```python
from build123d import *

# Parameters (mm, degrees)
SKETCH1_R           = 13
SKETCH1_R_2         = 6.25
BOSS_EXTRUDE1_DEPTH = 9


with BuildPart() as part:
    # Sketch1 → Boss-Extrude1 (new body)
    with BuildSketch(Plane(origin=(0, 0, 0), x_dir=(1, 0, 0), z_dir=(0, 1, 0))):
        with BuildLine():
            Line((2.928932188, 22.071067812), (22.071067812, 2.928932188))
            ThreePointArc((22.071067812, 2.928932188), (25.3153013, 0.761204675), (29.142135624, 0))
            Line((29.142135624, 0), (43, 0))
            ThreePointArc((43, 0), (57.142135624, 5.857864376), (63, 20))
            Line((63, 20), (63, 212))
            ThreePointArc((63, 212), (57.142135624, 226.142135624), (43, 232))
            Line((43, 232), (25, 232))
            ThreePointArc((25, 232), (10.857864376, 226.142135624), (5, 212))
            Line((5, 212), (5, 72.571067812))
            ThreePointArc((5, 72.571067812), (4.619397663, 70.65765065), (3.535533906, 69.035533906))
            Line((3.535533906, 69.035533906), (1.464466094, 66.964466094))
            ThreePointArc((1.464466094, 66.964466094), (0.380602337, 65.34234935), (0, 63.428932188))
            Line((0, 63.428932188), (0, 29.142135624))
            ThreePointArc((0, 29.142135624), (0.761204675, 25.3153013), (2.928932188, 22.071067812))
        make_face()
        with Locations(Location((38, 25, 0), (0, 0, 270))):
            Circle(SKETCH1_R, mode=Mode.SUBTRACT)
        with Locations(Location((38, 207, 0), (0, 0, 270))):
            Circle(SKETCH1_R, mode=Mode.SUBTRACT)
        with Locations(Location((26.5, 166.5, 0), (0, 0, 270))):
            Circle(SKETCH1_R_2, mode=Mode.SUBTRACT)
    extrude(amount=BOSS_EXTRUDE1_DEPTH)


solid = part.part
```
Could you check a few things on this model? Use its own coordinates, in mm. Give positions to 0.01 mm unless a question says otherwise; leave off trailing zeros. Loops run counter-clockwise (first coordinate to the right, second up) from the corner with the lowest first, then second, coordinate; pieces in that order, holes last. Notation, with made-up numbers: (-15, 71.25) -> (8, 71.25) arc R36 cw to (8, 110.25) -> close; hole circle Ø1 at (-29, -6.75). An arc over 180 degrees is marked (long way). Put each result on its own line as item: value.
(1) Thinking about a two-plate mould opening in X: for faces 1 (the face through (5, 4, -143)), 2 (the face through (57.297, 4.437, -225.986)), 3 (the face through (41.9, 4.4, -194.6)), which applies, pulls with the +X half, pulls with the -X half, needs draft (parallel to the pull), parting line crosses it, or undercut?
Computed:
face 1: pulls with the -X half
face 2: pulls with the +X half
face 3: undercut
(2) Imagine slicing it at C-C on y = 5.25. Write out the boundary of the cut face in (x, z), plus the area to 3 significant figures.
Computed:
outline: (0, -63.43) arc R5 ccw to (1.46, -66.96) -> (3.54, -69.04) arc R5 cw to (5, -72.57) -> (5, -212) arc R20 ccw to (25, -232) -> (43, -232) arc R20 ccw to (63, -212) -> (63, -20) arc R20 ccw to (43, 0) -> (29.14, 0) arc R10 ccw to (22.07, -2.93) -> (2.93, -22.07) arc R10 ccw to (0, -29.14) -> close; hole circle Ø12.5 at (26.5, -166.5); hole circle Ø26 at (38, -207); hole circle Ø26 at (38, -25)
area: 12,000 mm^2
(3) Imagine slicing it at A-A on x = 38. Write out the boundary of the cut face in (y, z).
Computed:
outline: (0, -232) -> (9, -232) -> (9, -220) -> (0, -220) -> close; (0, -194) -> (9, -194) -> (9, -38) -> (0, -38) -> close; (0, -12) -> (9, -12) -> (9, 0) -> (0, 0) -> close
(4) Imagine slicing it at B-B on z = -166.5. Write out the boundary of the cut face in (x, y), plus the area to 4 significant figures.
Computed:
outline: (5, 0) -> (20.25, 0) -> (20.25, 9) -> (5, 9) -> close; (32.75, 0) -> (63, 0) -> (63, 9) -> (32.75, 9) -> close
area: 409.5 mm^2
(5) Please list where these lines run through material, in increasing order: probe 1 along Z at (x, y) = (39, 5.5); probe 2 along Z at (x, y) = (27.5, 5.75); probe 3 along Z at (x, y) = (29.5, 5). Write a range as [from, to].
Computed:
probe 1: [-232, -219.96], [-194.04, -37.96], [-12.04, 0]
probe 2: [-232, -214.66], [-199.34, -172.67], [-160.33, -32.66], [-17.34, -0.14]
probe 3: [-232, -216.84], [-197.16, -171.98], [-161.02, -34.84], [-15.16, 0]
(6) Imagine slicing it at D-D on z = -207. Write out the boundary of the cut face in (x, y).
Computed:
outline: (5, 0) -> (25, 0) -> (25, 9) -> (5, 9) -> close; (51, 0) -> (63, 0) -> (63, 9) -> (51, 9) -> close
(7) I'm going to push flat-ended pins straight in: pin 1 Ø5 at (y, z) = (7, -26) entering from -X; pin 2 Ø3 at (x, y) = (14.5, 8) entering from -Z; pin 3 Ø4 at (x, y) = (13, 5) entering from +Z; pin 4 Ø15.5 at (x, z) = (38, -25) entering from +Y. Where does each tip first touch, or does it pass through?
Computed:
pin 1: x = 0.02
pin 2: z = -229.86
pin 3: z = -10
pin 4: through
